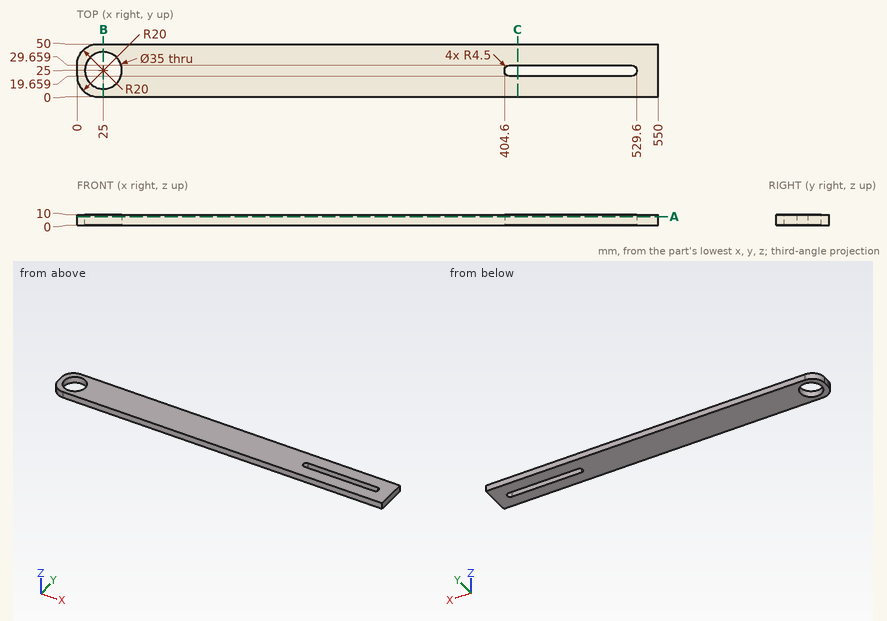
For this review, use the dimensioned drawing (mm, ordinates from the lowest corner) and the shaded views. Coordinates: 2 decimals unless noted, no trailing zeros. Loops run counter-clockwise (first coordinate to the right, second up) from the corner with the lowest first, then second, coordinate; pieces in that order, holes last. Notation, with made-up numbers: (28, 67) -> (53, 67) arc R33 cw to (53, 104) -> close; hole circle Ø2 at (-3, -40). An arc over 180 degrees is marked (long way). Write each question's results on one line, items separated by ' | '.
Q1. To check wall thickness, follow line 1 along X through (y, z) = (23.5, 3.5); line 2 along Y through (x, z) = (25, 3.75); line 3 along X through (y, z) = (21.5, 2). State the ranges of each line that lie inside material, in increasing order. Write a range as [from, to].
Taken from the geometry:
line 1: [0, 7.56], [42.44, 404.65], [529.55, 550] | line 2: [0, 7.5], [42.5, 50] | line 3: [0, 7.85], [42.15, 405.47], [528.73, 550]
Q2. For pin 1 Ø10 at (x, y) = (404.5, 41.5) entering from -Z, flat-tipped, find the tip position at first contact; note if it passes through.
Taken from the geometry:
pin 1: z = 0
Q3. Add section A-A, the plane z = 8.25. State the section outline as (x, y) points.
Taken from the geometry:
outline: (0, 20) arc R20 ccw to (20, 0) -> (550, 0) -> (550, 50) -> (20, 50) arc R20 ccw to (0, 30) -> close; hole circle Ø35 at (25, 25); hole (404.6, 24.16) arc R4.5 ccw to (409.1, 19.66) -> (525.1, 19.66) arc R4.5 ccw to (529.6, 24.16) -> (529.6, 25.16) arc R4.5 ccw to (525.1, 29.66) -> (409.1, 29.66) arc R4.5 ccw to (404.6, 25.16) -> close
Q4. Add section C-C, the plane x = 417. State the section outline as (y, z) points.
Taken from the geometry:
outline: (0, 0) -> (19.66, 0) -> (19.66, 10) -> (0, 10) -> close; (29.66, 0) -> (50, 0) -> (50, 10) -> (29.66, 10) -> close
Q5. Add section B-B, the plane x = 25. State the section outline as (y, z) points, then the cut area to 3 significant figures.
Taken from the geometry:
outline: (0, 0) -> (7.5, 0) -> (7.5, 10) -> (0, 10) -> close; (42.5, 0) -> (50, 0) -> (50, 10) -> (42.5, 10) -> close | area: 150 mm²
